```python
from build123d import *

# Parameters (mm, degrees)
BOSS_EXTRUDE1_DEPTH = 2
SKETCH2_R           = 2.85029491
SKETCH2_R_2         = 2
BOSS_EXTRUDE2_DEPTH = 4
SKETCH3_R           = 0.75
SKETCH3_R_2         = 1.25
CUT_EXTRUDE1_DEPTH  = 10


with BuildPart() as part:
    # Sketch1 → Boss-Extrude1 (new body)
    with BuildSketch(Plane(origin=(0, 0, 0), x_dir=(1, 0, 0), z_dir=(0, 1, 0))):
        with BuildLine():
            Line((0, 2.85029491), (20, 1.5))
            ThreePointArc((20, 1.5), (21.5, 0), (20, -1.5))
            Line((20, -1.5), (0, -2.85029491))
            ThreePointArc((0, -2.85029491), (-2.85029491, 0), (0, 2.85029491))
        make_face()
    extrude(amount=BOSS_EXTRUDE1_DEPTH)

    # Sketch2 → Boss-Extrude2 (add)
    with BuildSketch(Plane(origin=(0, 2, 0), x_dir=(1, 0, 0), z_dir=(0, 1, 0))):
        with Locations(Location((0, 0, 0), (0, 0, 270))):
            Circle(SKETCH2_R)
        with Locations(Location((0, 0, 0), (0, 0, 270))):
            Circle(SKETCH2_R_2, mode=Mode.SUBTRACT)
    extrude(amount=BOSS_EXTRUDE2_DEPTH)

    # Sketch3 → Cut-Extrude1 (cut)
    with BuildSketch(Plane.XZ):
        with Locations(Location((16, 0, 0), (0, 0, 270))):
            Circle(SKETCH3_R)
        with Locations(Location((12, 0, 0), (0, 0, 270))):
            Circle(SKETCH3_R)
        with Locations(Location((7, 0, 0), (0, 0, 270))):
            Circle(SKETCH3_R_2)
        with Locations(Location((20, 0, 0), (0, 0, 270))):
            Circle(SKETCH3_R)
    extrude(amount=-CUT_EXTRUDE1_DEPTH, mode=Mode.SUBTRACT)


solid = part.part
```
Could you check a few things on this model? Use its own coordinates, in mm. A direction names the side the tool comes from. Give positions to 0.01 mm unless a question says otherwise; leave off trailing zeros. Order: outer loops, then holes, each group sorted by start corner. A loop starts at its lowest first (then second) coordinate and runs counter-clockwise, first axis right, second up.
Q1. If I drill on line 1 along X through (y, z) = (1.55, 0); line 2 along Y through (x, z) = (17.75, -0.7); line 3 along X through (y, z) = (0.75, -1.05), over which ranges is the centre line in solid material (lowest first)?
Q2. Suppose I cut it at B-B, the plane y = 1.45. Write out the boundary of the cut face in (x, z).
Q3. We'd pull the mould along Z, two halves only. Please class faces 1 (the flat face through (11, 2, 0)), 2 (the cylindrical face through (-2.529, 3.625, 1.315)), 3 (the flat face through (10.14, 0.986, 2.166)), 4 (the cylindrical face through (-2, 4, 0)): +Z half, -Z half, draft (parallel to the pull), parting line (faces both ways), or undercut.
Q4. Suppose I cut it at A-A, the plane z = 0. Write out the boundary of the cut face in (x, y), and give its area (3 significant figures).
Q5. I'm going to push a flat-ended pin straight in: P1, Ø1.2, axis at x = 0.5, z = -0.5, coming from the +Y side. Where does the tip first touch, or does it pass through?
Q6. For faces 5 (the flat face through (2, 6, 1)), 6 (the flat face through (0, 2, 0)), which set-ups out of +Z, -Z, +X, -X, +Y, -Y let a thin tool reach every point of the face, with its end or its side?
Q7. Suppose I cut it at C-C, the plane x = 16. Write out the boundary of the cut face in (y, z).
Q8. Suppose I cut it at D-D, the plane x = -0.75. Write out the boundary of the cut face in (y, z), and give its area (3 significant figures).
Solution:
1. line 1: x = -2.85 to 5.75, 8.25 to 11.25, 12.75 to 15.25, 16.75 to 19.25, 20.75 to 21.5
1. line 2: y = 0 to 2
1. line 3: x = -2.65 to 6.32, 7.68 to 21.07
2. outline: (0, -2.85) - (20, -1.5) arc R1.5 ccw to (20, 1.5) - (0, 2.85) arc R2.85 ccw to start; hole circle Ø2.5 at (7, 0); hole circle Ø1.5 at (12, 0); hole circle Ø1.5 at (16, 0); hole circle Ø1.5 at (20, 0)
3. face 1: draft
3. face 2: parting line
3. face 3: +Z half
3. face 4: undercut
4. outline: (-2.85, 0) - (5.75, 0) - (5.75, 2) - (2.85, 2) - (2.85, 6) - (2, 6) - (2, 2) - (-2, 2) - (-2, 6) - (-2.85, 6) - close; (8.25, 0) - (11.25, 0) - (11.25, 2) - (8.25, 2) - close; (12.75, 0) - (15.25, 0) - (15.25, 2) - (12.75, 2) - close; (16.75, 0) - (19.25, 0) - (19.25, 2) - (16.75, 2) - close; (20.75, 0) - (21.5, 0) - (21.5, 2) - (20.75, 2) - close
4. area: 41.5 mm2
5. P1: stops at y = 2
6. face 5: +Z, -Z, +X, -X, +Y
6. face 6: +Y
7. outline: (0, -1.77) - (2, -1.77) - (2, -0.75) - (0, -0.75) - close; (0, 0.75) - (2, 0.75) - (2, 1.77) - (0, 1.77) - close
8. outline: (0, -2.75) - (6, -2.75) - (6, -1.85) - (2, -1.85) - (2, 1.85) - (6, 1.85) - (6, 2.75) - (0, 2.75) - close
8. area: 18.2 mm2
